The figure shows three views and two pictorial views of one solid part (mm, origin at its lowest corner). Answer the questions. Give positions to 0.01 mm unless a question says otherwise; leave off trailing zeros. Order: outer loops, then holes, each group sorted by start corner. A loop starts at its lowest first (then second) coordinate and runs counter-clockwise, first axis right, second up. Notation, with made-up numbers: (-24.75, 64.25) - (33.25, 64.25) arc R28 cw to (33.25, 85.25) - close; hole circle Ø1 at (62, -12). An arc over 180 degrees is marked (long way). Answer as CSV lines item,"result". Start each with the question number.
1. Section A-A on x = 10 is taken. Give the vertices of the cut face in (y, z), and give its area (3 significant figures).
2. Section B-B on z = 12 is taken. Give the vertices of the cut face in (x, y), and give its area (3 significant figures).
3. A flat-ended cylindrical pin translates along its axis: pin 1 (6 mm diameter, centred on x = 60, z = 12, fed in from -Y). Find the tip coordinate at first contact, or state that the pin passes through.
4. Consider line 1 along X through (y, z) = (8.5, 188); line 2 along Z through (x, y) = (10, 3.5); line 3 along Z through (x, y) = (9, 6.25). Determine where each line is inside the solid, lowest interval first. Write a range as [from, to].
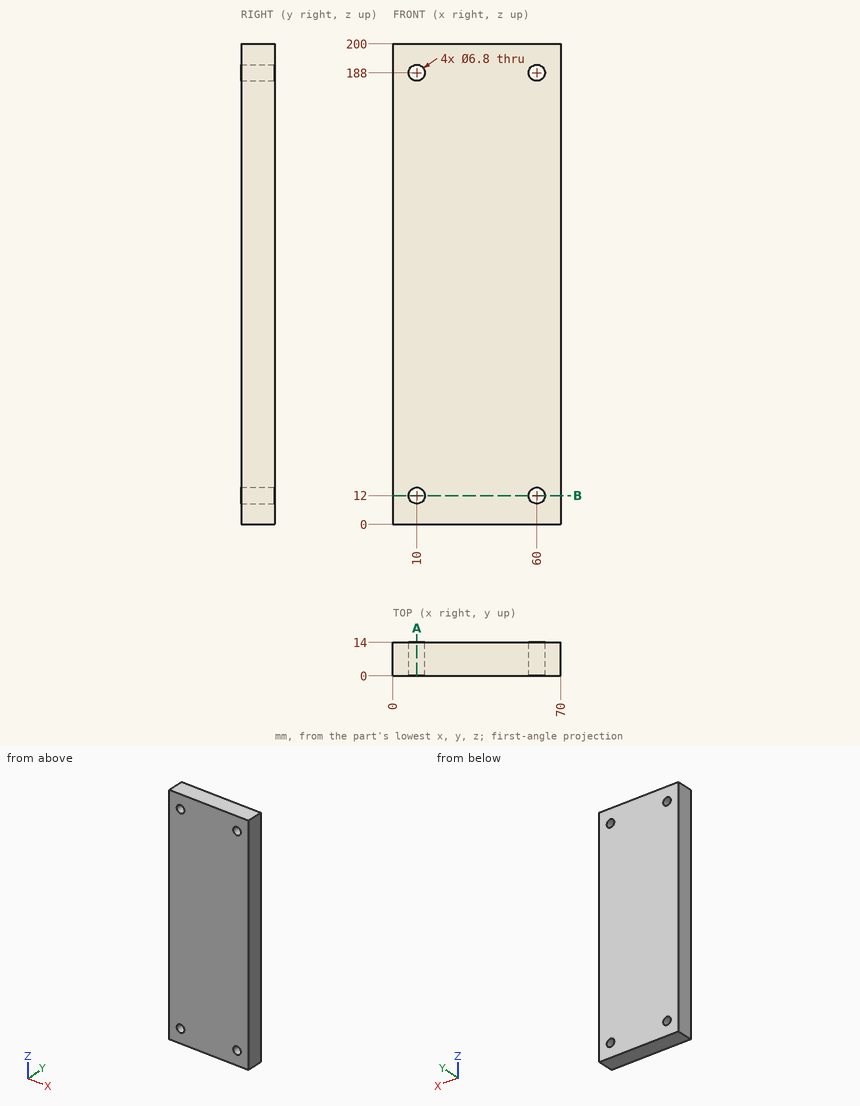
Checks:
1,outline,"(0, 0) - (14, 0) - (14, 8.6) - (0, 8.6) - close; (0, 15.4) - (14, 15.4) - (14, 184.6) - (0, 184.6) - close; (0, 191.4) - (14, 191.4) - (14, 200) - (0, 200) - close"
1,area,"2,610 mm²"
2,outline,"(0, 0) - (6.6, 0) - (6.6, 14) - (0, 14) - close; (13.4, 0) - (56.6, 0) - (56.6, 14) - (13.4, 14) - close; (63.4, 0) - (70, 0) - (70, 14) - (63.4, 14) - close"
2,area,"790 mm²"
3,pin 1,"passes through"
4,line 1,"x = [0, 6.6], [13.4, 56.6], [63.4, 70]"
4,line 2,"z = [0, 8.6], [15.4, 184.6], [191.4, 200]"
4,line 3,"z = [0, 8.75], [15.25, 184.75], [191.25, 200]"
